```python
from build123d import *

# Parameters (mm, degrees)
CLAMP_RING_PROFILE_R       = 48
CLAMP_RING_96_DEPTH        = 20
END_BOSS_PROFILE_R         = 26
END_BOSS_52_DEPTH          = 20
LEVER_WEB_DEPTH            = 40
RIB_A_DEPTH                = 6
RIB_B_DEPTH                = 6
CLAMP_BORE_PROFILE_R       = 32
CLAMP_BORE_DEPTH           = 213
END_BORE_PROFILE_R         = 14
END_BORE_DEPTH             = 213
CLAMP_LUG_DEPTH            = 40
CLAMP_SLOT_DEPTH           = 40
CLAMP_SCREW_HOLE_PROFILE_R = 5
CLAMP_SCREW_HOLE_DEPTH     = 105


with BuildPart() as part:
    # Clamp Ring Profile → Clamp Ring Ø96 (new, symmetric)
    with BuildSketch(Plane.XY):
        Circle(CLAMP_RING_PROFILE_R)
    extrude(amount=CLAMP_RING_96_DEPTH, both=True)



with BuildPart() as body_2:
    # End Boss Profile → End Boss Ø52 (new, symmetric)
    with BuildSketch(Plane.XY):
        with Locations((110, 0)):
            Circle(END_BOSS_PROFILE_R)
    extrude(amount=END_BOSS_52_DEPTH, both=True)


with BuildPart() as part_1:
    add(part.part)

    add(body_2.part)  # Lever Web merges body 2
    # Lever Web Profile → Lever Web (add)
    with BuildSketch(Plane.XY.offset(20)):
        Polygon((48, 6), (86.790548166, 6), (86.790548166, -6), (44, -6), (44, 6), align=None)
    extrude(amount=-LEVER_WEB_DEPTH)

    # Rib A Profile → Rib A (add, symmetric)
    with BuildSketch(Plane.XY):
        with BuildLine():
            Line((110, 26), (40.348482004, 26))
            ThreePointArc((40.348482004, 26), (45.108407669, 16.408277105), (47.623523599, 6))
            Line((47.623523599, 6), (84.701778719, 6))
            ThreePointArc((84.701778719, 6), (93.875484503, 20.396078054), (110, 26))
        make_face()
    extrude(amount=RIB_A_DEPTH, both=True)

    # Rib B Profile → Rib B (add, symmetric)
    with BuildSketch(Plane.XY):
        with BuildLine():
            Line((110, -26), (40.276028999, -26))
            ThreePointArc((40.276028999, -26), (45.014976817, -16.391327753), (47.623523599, -6))
            Line((47.623523599, -6), (84.701778719, -6))
            ThreePointArc((84.701778719, -6), (93.875484503, -20.396078054), (110, -26))
        make_face()
    extrude(amount=RIB_B_DEPTH, both=True)

    # Clamp Bore Profile → Clamp Bore (cut)
    with BuildSketch(Plane.XY.offset(20)):
        Circle(CLAMP_BORE_PROFILE_R)
    extrude(amount=-CLAMP_BORE_DEPTH, mode=Mode.SUBTRACT)

    # End Bore Profile → End Bore (cut)
    with BuildSketch(Plane.XY.offset(20)):
        with Locations((110, 0)):
            Circle(END_BORE_PROFILE_R)
    extrude(amount=-END_BORE_DEPTH, mode=Mode.SUBTRACT)

    # Clamp Lug Profile → Clamp Lug (add)
    with BuildSketch(Plane.XY.offset(20)):
        Polygon((0, -37.46998799), (30, -37.46998799), (30, -67.46998799), (-30, -67.46998799), (-30, -37.46998799), align=None)
    extrude(amount=-CLAMP_LUG_DEPTH)

    # Clamp Slot Profile → Clamp Slot (cut)
    with BuildSketch(Plane.XY.offset(20)):
        Polygon((0, -67.46998799), (3, -67.46998799), (3, -25.366050336), (-3, -25.366050336), (-3, -67.46998799), align=None)
    extrude(amount=-CLAMP_SLOT_DEPTH, mode=Mode.SUBTRACT)

    # Clamp Screw Hole Profile → Clamp Screw Hole (cut)
    with BuildSketch(Plane(origin=(30, 0, 0), x_dir=(0, 0, -1), z_dir=(1, 0, 0))):
        with Locations(Location((0, -53.46998799, 0), (0, 0, 90))):
            Circle(CLAMP_SCREW_HOLE_PROFILE_R)
    extrude(amount=-CLAMP_SCREW_HOLE_DEPTH, mode=Mode.SUBTRACT)


solid = part_1.part
```
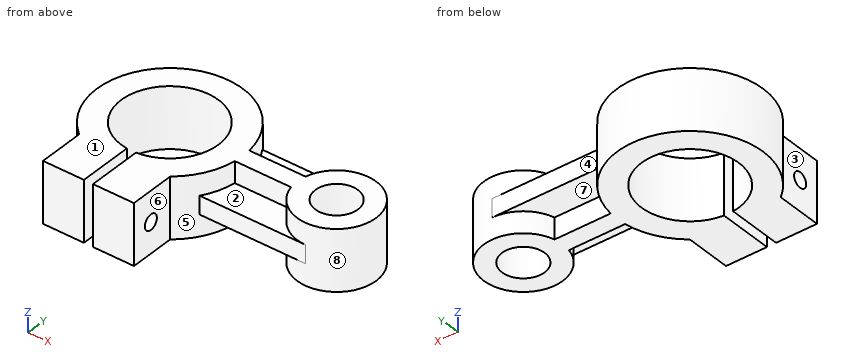
The listing builds one solid part. Answer for the finished solid, in the listing's coordinates (mm). Face numbers are marked on the shaded views. A direction names the side the tool comes from. Coordinates: 2 decimals unless noted, no trailing zeros. Loops run counter-clockwise (first coordinate to the right, second up) from the corner with the lowest first, then second, coordinate; pieces in that order, holes last. Notation, with made-up numbers: (12.25, -21) - (55.25, -21) arc R15 ccw to (55.25, -6) - close; hole circle Ø10 at (71, 31.5). An arc over 180 degrees is marked (long way). Write item = value, one per line.
1) Section C-C (z = 8) is taken. Determine the outline of the cut face in (x, y), plus the area to 3 significant figures.
Responses:
outline = (-30, -67.47) - (-3, -67.47) - (-3, -31.86) arc R32 cw (long way) to (3, -31.86) - (3, -67.47) - (30, -67.47) - (30, -37.47) arc R48 ccw to (47.62, -6) - (84.7, -6) arc R26 ccw (long way) to (84.7, 6) - (47.62, 6) arc R48 ccw (long way) to (-30, -37.47) - close; hole circle Ø28 at (110, 0)
area = 7,120 mm^2
2) Section A-A (z = 0) is taken. Determine the outline of the cut face in (x, y), plus the area to 3 significant figures.
Responses:
outline = (-30, -67.47) - (-3, -67.47) - (-3, -58.47) - (-30, -58.47) - close; (-30, -48.47) - (-3, -48.47) - (-3, -31.86) arc R32 cw (long way) to (3, -31.86) - (3, -48.47) - (30, -48.47) - (30, -37.47) arc R48 ccw to (40.35, -26) - (110, -26) arc R26 ccw to (110, 26) - (40.35, 26) arc R48 ccw (long way) to (-30, -37.47) - close; (3, -67.47) - (30, -67.47) - (30, -58.47) - (3, -58.47) - close; hole circle Ø28 at (110, 0)
area = 8,430 mm^2
3) Which of the six approach directions +Z, -Z, +X, -X, +Y, -Y give full straight-line access (tool end or side, diameter ignored) to the marked faces 4, 5, 6, 7 and 8?
Responses:
face_4 = +Z, -Z, +X, +Y
face_5 = -Y
face_6 = +Z, -Z, +X, -Y
face_7 = -Z, +Y
face_8 = none
4) Find the intervals of material crossed by line 1 along X through (y, z) = (-44, 17); line 2 along X through (y, z) = (10.5, 13.5); line 3 along Y through (x, z) = (-11, -0.5), in increasing order.
Responses:
line_1 = -30 to -3, 3 to 30
line_2 = -46.84 to -30.23, 30.23 to 46.84, 86.21 to 100.74, 119.26 to 133.79
line_3 = -67.47 to -58.44, -48.5 to -30.05, 30.05 to 46.72
5) Section B-B (x = 6) is taken. Determine the outline of the cut face in (y, z), plus the area to 3 significant figures.
Responses:
outline = (-67.47, -20) - (-31.43, -20) - (-31.43, 20) - (-67.47, 20) - close; (31.43, -20) - (47.62, -20) - (47.62, 20) - (31.43, 20) - close; hole circle Ø10 at (-53.47, 0)
area = 2,010 mm^2
6) Determine the mould class of the marked faces 1, 2 and 3 for opening direction X: pulls with the +X half, pulls with the -X half, needs draft (parallel to the pull), parting line crosses it, or undercut.
Responses:
face_1 = needs draft
face_2 = undercut
face_3 = pulls with the -X half
7) Each of these flat-tipped pins is pushed along its axis until it touches: P1, Ø2, axis at y = -38.5, z = 1, coming from the -X side; P2, Ø10, axis at x = 76.5, y = 20.5, coming from the +Z side; P3, Ø10.5, axis at y = -42.5, z = -9, coming from the +X side. Where does it stop, or does it pass through?
Responses:
P1 = -30
P2 = 6
P3 = 30.27
8) Section D-D (x = 66) is taken. Determine the outline of the cut face in (y, z), plus the area to 3 significant figures.
Responses:
outline = (-26, -6) - (-6, -6) - (-6, -20) - (6, -20) - (6, -6) - (26, -6) - (26, 6) - (6, 6) - (6, 20) - (-6, 20) - (-6, 6) - (-26, 6) - close
area = 960 mm^2
